Could you check a few things on this drawing? It's one solid part, dimensions in mm from its lowest x, y, z. A direction names the side the tool comes from. Give positions to 0.01 mm unless a question says otherwise; leave off trailing zeros. Order: outer loops, then holes, each group sorted by start corner. A loop starts at its lowest first (then second) coordinate and runs counter-clockwise, first axis right, second up. Notation, with made-up numbers: (32.25, 71) - (42.25, 71) arc R24 ccw to (42.25, 96) - close; hole circle Ø9 at (17.25, -16.5). An arc over 180 degrees is marked (long way). Put each result on its own line as item: value.
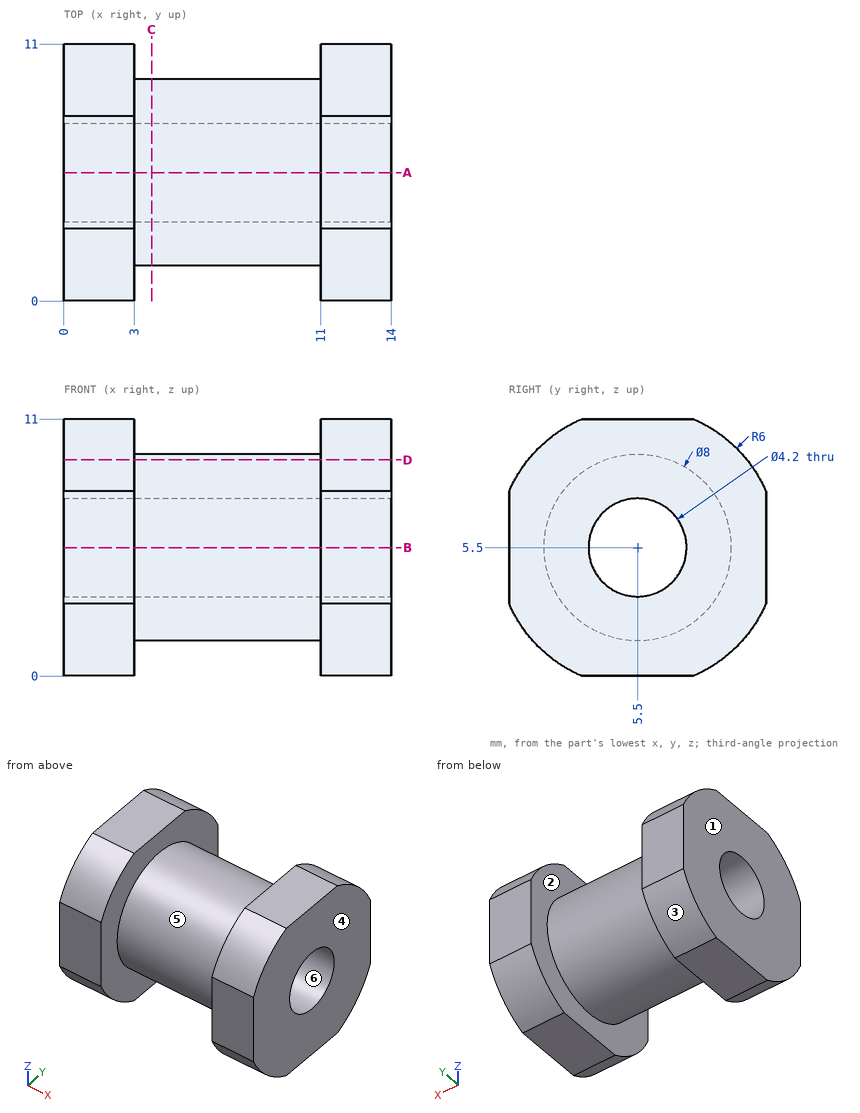
1) We'd pull the mould along X, two halves only. Please class the marked faces 1, 2, 3 and 4: pulls with the +X half, pulls with the -X half, needs draft (parallel to the pull), parting line crosses it, or undercut.
Filled in:
face 1: pulls with the -X half
face 2: undercut
face 3: needs draft
face 4: pulls with the +X half
2) If I drill on line 1 (X direction, y = 9, z = 8.25); line 2 (Y direction, x = 9.25, z = 4.75); line 3 (Y direction, x = 12.5, z = 5), over which ranges is the centre line in solid material (lowest first)? Write a range as [from, to].
Filled in:
line 1: x = [0, 3], [11, 14]
line 2: y = [1.57, 3.54], [7.46, 9.43]
line 3: y = [0, 3.46], [7.54, 11]
3) Suppose I cut it at D-D, the plane z = 9.25. List the corners of the cut face in (x, y) for me.
Filled in:
outline: (0, 0.82) - (3, 0.82) - (3, 4.11) - (11, 4.11) - (11, 0.82) - (14, 0.82) - (14, 10.18) - (11, 10.18) - (11, 6.89) - (3, 6.89) - (3, 10.18) - (0, 10.18) - close
4) Suppose I cut it at C-C, the plane x = 3.75. List the corners of the cut face in (y, z) for me, and give its area (3 significant figures).
Filled in:
outline: circle Ø8 at (5.5, 5.5); hole circle Ø4.2 at (5.5, 5.5)
area: 36.4 mm^2
5) Suppose I cut it at A-A, the plane y = 5.5. List the corners of the cut face in (x, z) for me.
Filled in:
outline: (0, 0) - (3, 0) - (3, 1.5) - (11, 1.5) - (11, 0) - (14, 0) - (14, 3.4) - (0, 3.4) - close; (0, 7.6) - (14, 7.6) - (14, 11) - (11, 11) - (11, 9.5) - (3, 9.5) - (3, 11) - (0, 11) - close
6) Which directions (+Z, -Z, +X, -X, +Y, -Y) give clear straight access to the entire face, cutting with the end or side of a thin tool? Please do the marked faces 5 and 6.
Filled in:
face 5: none
face 6: +X, -X
7) I'm going to push flat-ended pins straight in: pin 1 (3 mm diameter, centred on y = 6.5, z = 7, fed in from -X); pin 2 (1 mm diameter, centred on x = 5.5, y = 2.5, fed in from -Z); pin 3 (4 mm diameter, centred on x = 7, z = 4.5, fed in from -Y); pin 4 (1.5 mm diameter, centred on x = 9.5, y = 2, fed in from +Z). Where does each tip first touch, or does it pass through?
Filled in:
pin 1: stops at x = 0
pin 2: stops at z = 2.38
pin 3: stops at y = 1.5
pin 4: stops at z = 8.4
